The model under review builds one solid part; all positions refer to its coordinate system, in mm. Round coordinates to 2 decimals unless told otherwise and drop trailing zeros. Write each loop counter-clockwise with the first axis right and the second up, starting at its lowest first coordinate (ties: lowest second). Pieces come first, ordered by that corner, then holes. Notation, with made-up numbers: M 88,-35.75 L 103,-35.75 A17 cw 103,-30.75 Z; hole C 5.25,24.5 d2. An arc over 180 degrees is marked long. Write item = value, one per line. Start each with the question number.
Item 1: To check wall thickness, follow line 1 along Y through (x, z) = (-88, 4.15); line 2 along Y through (x, z) = (8, 3.15); line 3 along Y through (x, z) = (46.5, 0.65). State the ranges of each line that lie inside material, in increasing order.
Item 2: Take a section at D-D, the plane y = 55. Give the boundary of the cut face in (x, z).
Item 3: Take a section at A-A, the plane y = -62.5. Give the boundary of the cut face in (x, z).
Item 4: The part is to be moulded in two halves that separate along X. For faces 1 (the cylindrical face through (-43.708, -61.148, 3.042)), 2 (the flat face through (-103, -1, 3)), 3 (the flat face through (-1, 1, 0)), say which applies: +X half, -X half, draft (parallel to the pull), parting line (faces both ways), or undercut.
Item 5: Take a section at C-C, the plane z = 1.5. Give the number of separate pieces and of enclosed holes in the cut face, plus the area to 3 significant figures.
Item 6: For pin 1 Ø6 at (x, y) = (84, 15.5) entering from -Z, flat-tipped, find the tip position at first contact; note if it passes through.
Item 7: Take a section at B-B, the plane x = -88. Give the boundary of the cut face in (y, z).
from build123d import *

# Parameters (mm, degrees)
SKETCH_1_W               = 206
SKETCH_1_H               = 145
EXTRUDE_1_DEPTH          = 6
SKETCH_3_R               = 4.5
CUT_EXTRUDE_2_DEPTH      = 127.100158604
SKETCH_4_R               = 15
CUT_EXTRUDE_3_DEPTH      = 127.100158604
FILLET_1_R               = 57
HOLE_WIZARD_M8_1_D       = 6.8
PATTERN_CIRCULAR_1_COUNT = 2
SKETCH_11_R              = 4.5
CUT_EXTRUDE_6_DEPTH      = 127.100158604
FILLET_5_R               = 3


with BuildPart() as part:
    # 草图1 → 凸台-拉伸1 (new body)
    with BuildSketch(Plane.XY):
        Rectangle(SKETCH_1_W, SKETCH_1_H)
    extrude(amount=EXTRUDE_1_DEPTH)

    # 草图3 → 切除-拉伸2 (cut, through all)
    with BuildSketch(Plane.XY.offset(6)):
        with Locations((-88, 55)):
            Circle(SKETCH_3_R)
        with Locations((-48, 55)):
            Circle(SKETCH_3_R)
        with Locations((-88, -62.5)):
            Circle(SKETCH_3_R)
        with Locations((-48, -62.5)):
            Circle(SKETCH_3_R)
    extrude(amount=-CUT_EXTRUDE_2_DEPTH, mode=Mode.SUBTRACT)

    # 草图4 → 切除-拉伸3 (cut, through all)
    with BuildSketch(Plane.XY.offset(6)):
        with Locations((46, 15.5)):
            Circle(SKETCH_4_R)
    extrude(amount=-CUT_EXTRUDE_3_DEPTH, mode=Mode.SUBTRACT)

    # 圆角1
    fillet_1_edges = [part.edges().sort_by_distance(p)[0] for p in [
        (103, 72.5, 3),
    ]]
    fillet(fillet_1_edges, radius=FILLET_1_R)

    # M8 螺纹孔1 (through all)
    with Locations(Plane.XY.offset(6)):
        with Locations((8, 15.5)):
            hole_wizard_m8_1 = Hole(HOLE_WIZARD_M8_1_D / 2)

    # 阵列(圆周)1: M8 螺纹孔1 ×2 about axis
    pattern_circular_1_axis = Axis((46, 15.5, 0), (0, 0, 1))
    for i in range(1, PATTERN_CIRCULAR_1_COUNT):
        add(hole_wizard_m8_1.rotate(pattern_circular_1_axis, i * 360 / PATTERN_CIRCULAR_1_COUNT), mode=Mode.SUBTRACT)

    # 草图11 → 切除-拉伸6 (cut, through all)
    with BuildSketch(Plane.XY.offset(6)):
        with Locations((73, -62.5)):
            Circle(SKETCH_11_R)
    extrude(amount=-CUT_EXTRUDE_6_DEPTH, mode=Mode.SUBTRACT)

    # 圆角5
    fillet_5_edges = [part.edges().sort_by_distance(p)[0] for p in [
        (103, -72.5, 3),
    ]]
    fillet(fillet_5_edges, radius=FILLET_5_R)


solid = part.part
Response values:
q1.line_1 = -72.5 to -67, -58 to 50.5, 59.5 to 72.5
q1.line_2 = -72.5 to 12.1, 18.9 to 72.5
q1.line_3 = -72.5 to 0.51, 30.49 to 72.5
q2.outline = M -103,0 L -92.5,0 L -92.5,6 L -103,6 Z; M -83.5,0 L -52.5,0 L -52.5,6 L -83.5,6 Z; M -43.5,0 L 87.09,0 L 87.09,6 L -43.5,6 Z
q3.outline = M -103,0 L -92.5,0 L -92.5,6 L -103,6 Z; M -83.5,0 L -52.5,0 L -52.5,6 L -83.5,6 Z; M -43.5,0 L 68.5,0 L 68.5,6 L -43.5,6 Z; M 77.5,0 L 103,0 L 103,6 L 77.5,6 Z
q4.face_1 = undercut
q4.face_2 = -X half
q4.face_3 = draft
q5.separate_pieces = 1
q5.enclosed_holes = 8
q5.area = 28,100 mm2
q6.pin_1 = through
q7.outline = M -72.5,0 L -67,0 L -67,6 L -72.5,6 Z; M -58,0 L 50.5,0 L 50.5,6 L -58,6 Z; M 59.5,0 L 72.5,0 L 72.5,6 L 59.5,6 Z
